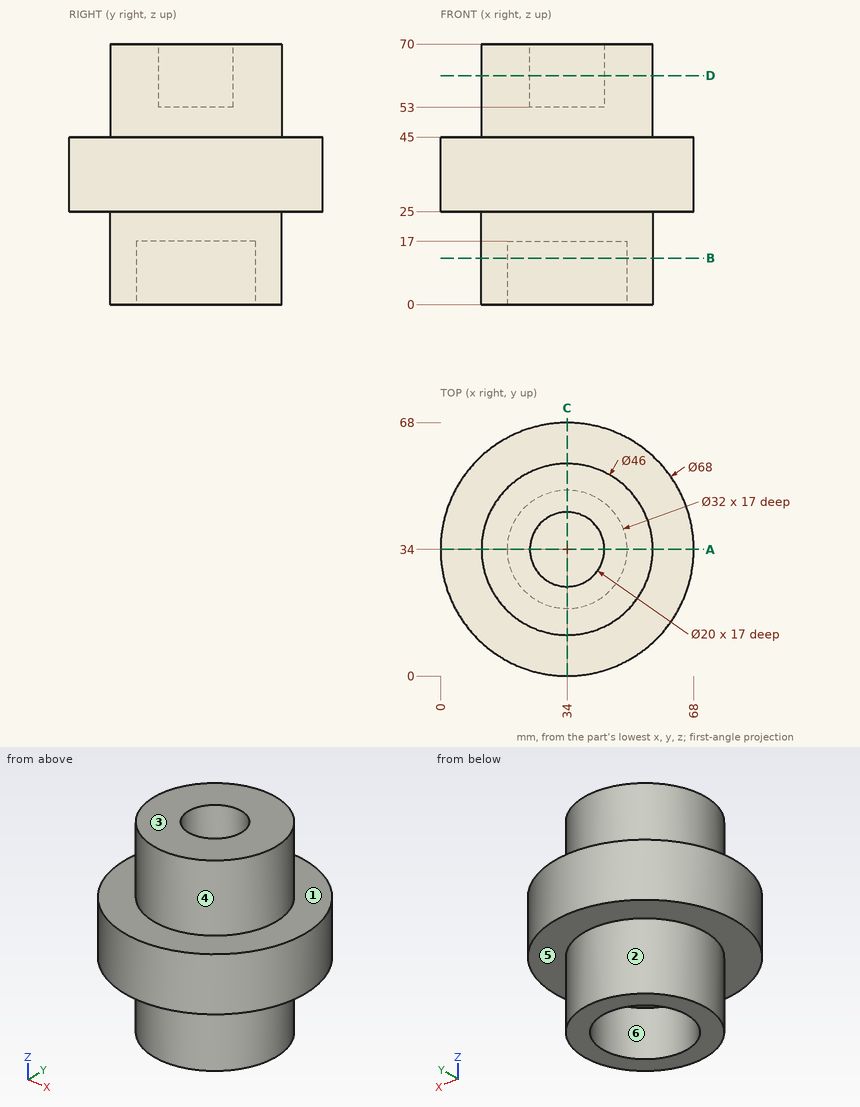
Drawing for the job (mm, zero at the part's lowest x, y, z). A direction names the side the tool comes from. Coordinates: 2 decimals unless noted, no trailing zeros. Loops run counter-clockwise (first coordinate to the right, second up) from the corner with the lowest first, then second, coordinate; pieces in that order, holes last. Notation, with made-up numbers: (-34, -1.75) - (-24, -1.75) arc R20 cw to (-24, 23.25) - close; hole circle Ø5 at (-31.75, 36). An arc over 180 degrees is marked (long way). Use CSV: the item, a comma, the result in double quotes. Start each with the question number.
Q1. Cut at A-A, the plane y = 34. List the corners of the cut face in (x, z), then the cut area to 3 significant figures.
Q2. Drop flat-ended pins along their axis: P1, Ø10, axis at x = 31, y = 30.5, coming from the +Z side; P2, Ø1, axis at x = 46.5, y = 59.5, coming from the -Z side; P3, Ø20.5, axis at x = 32.5, y = 33.5, coming from the -Z side; P4, Ø12, axis at x = 12.5, y = 51.5, coming from the -Z side. Give the stop position or say it passes through.
Q3. Cut at D-D, the plane z = 61.5. List the corners of the cut face in (x, y), then the cut area to 3 significant figures.
Q4. Probe probe 1 along Y at (x, z) = (34, 60.25); probe 2 along Y at (x, z) = (34, 13.75); probe 3 along Z at (x, y) = (47.5, 6.5). List the from-to ranges inside material, lowest first. Write a range as from..to.
Q5. Two-plate mould, pull along Y, no slides. Class the marked faces 4, 5 and 6: +Y half, -Y half, draft (parallel to the pull), parting line (faces both ways), or undercut.
Q6. Cut at B-B, the plane z = 12.5. List the corners of the cut face in (x, y), then the cut area to 3 significant figures.
Q7. 3-axis set-ups, long thin cutter, end or side, ignore diameter. For the marked faces 1, 2 and 3: which of +Z, -Z, +X, -X, +Y, -Y reach the whole face in a straight line?
Here are the results:
1,outline,"(0, 25) - (11, 25) - (11, 0) - (18, 0) - (18, 17) - (50, 17) - (50, 0) - (57, 0) - (57, 25) - (68, 25) - (68, 45) - (57, 45) - (57, 70) - (44, 70) - (44, 53) - (24, 53) - (24, 70) - (11, 70) - (11, 45) - (0, 45) - close"
1,area,"2,780 mm2"
2,P1,"z = 53"
2,P2,"z = 25"
2,P3,"z = 17"
2,P4,"z = 0"
3,outline,"circle Ø46 at (34, 34); hole circle Ø20 at (34, 34)"
3,area,"1,350 mm2"
4,probe 1,"11..24, 44..57"
4,probe 2,"11..18, 50..57"
4,probe 3,"25..45"
5,face 4,"parting line"
5,face 5,"draft"
5,face 6,"undercut"
6,outline,"circle Ø46 at (34, 34); hole circle Ø32 at (34, 34)"
6,area,"858 mm2"
7,face 1,"+Z"
7,face 2,"-Z"
7,face 3,"+Z, +X, -X, +Y, -Y"
